Could you check a few things on this drawing? It's one solid part, dimensions in mm from its lowest x, y, z. Give positions to 0.01 mm unless a question says otherwise; leave off trailing zeros. Order: outer loops, then holes, each group sorted by start corner. A loop starts at its lowest first (then second) coordinate and runs counter-clockwise, first axis right, second up. Notation, with made-up numbers: (88, -34.5) -> (101, -34.5) arc R35 cw to (101, 3.5) -> close; hole circle Ø6 at (34.5, 71). An arc over 180 degrees is marked (long way). Answer as CSV lines item,"result".
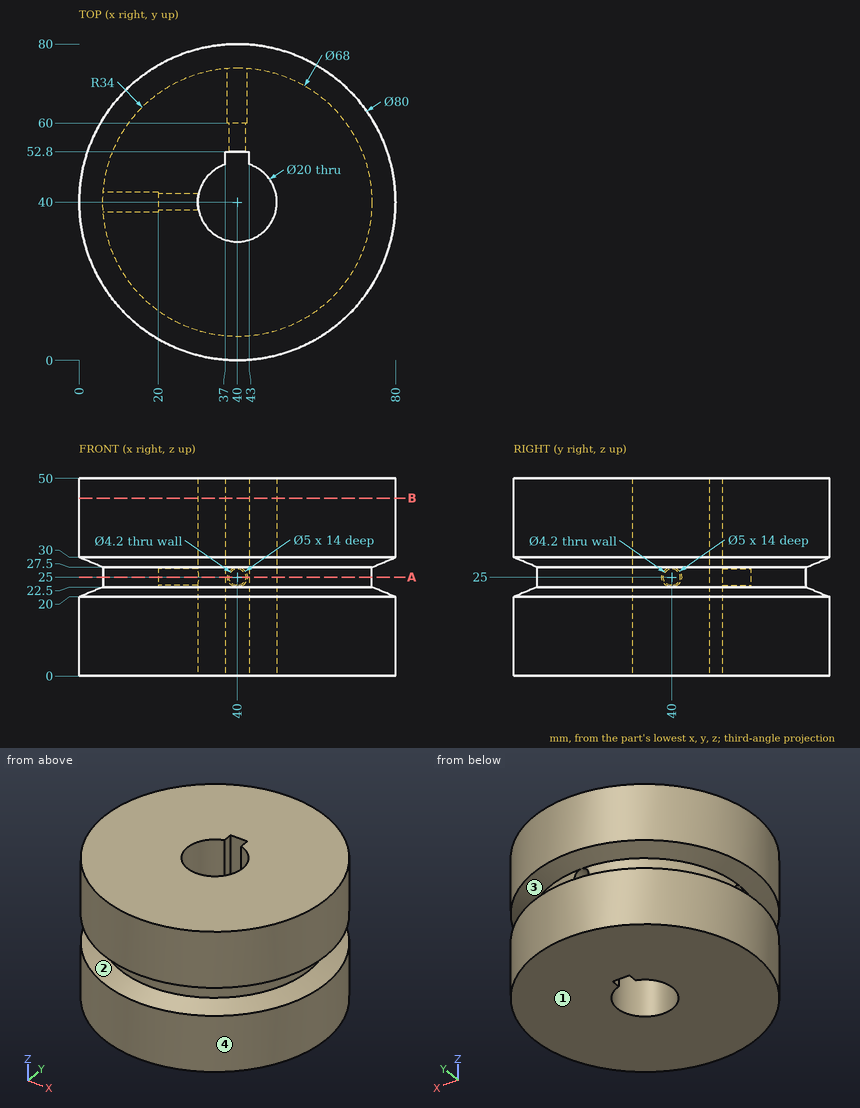
Item 1: Imagine slicing it at A-A, the plane z = 25. Please give me the cut outline in (x, y).
Numbers:
outline,"(6.09, 37.5) arc R34 ccw (long way) to (42.5, 73.91) -> (42.5, 60) -> (42.1, 60) -> (42.1, 52.8) -> (43, 52.8) -> (43, 49.54) arc R10 cw (long way) to (30.22, 37.9) -> (20, 37.9) -> (20, 37.5) -> close; (6.09, 42.5) -> (20, 42.5) -> (20, 42.1) -> (30.22, 42.1) arc R10 cw to (37, 49.54) -> (37, 52.8) -> (37.9, 52.8) -> (37.9, 60) -> (37.5, 60) -> (37.5, 73.91) arc R34 ccw to start"
Item 2: Imagine slicing it at B-B, the plane z = 45. Please give me the cut outline in (x, y).
Numbers:
outline,"circle Ø80 at (40, 40); hole (37, 49.54) arc R10 ccw (long way) to (43, 49.54) -> (43, 52.8) -> (37, 52.8) -> close"
Item 3: We'd pull the mould along Z, two halves only. Please class the marked faces 1, 2, 3 and 4: released by +Z, released by -Z, zero draft, split by the parting line, or undercut.
Numbers:
face 1,"released by -Z"
face 2,"undercut"
face 3,"undercut"
face 4,"zero draft"
Item 4: Please list where these lines run through material, in increasing order: line 1 along X through (y, z) = (40, 38.5); line 2 along Z through (x, y) = (40, 58); line 3 along Z through (x, y) = (40, 63).
Numbers:
line 1,"x = 0 to 30, 50 to 80"
line 2,"z = 0 to 22.9, 27.1 to 50"
line 3,"z = 0 to 22.5, 27.5 to 50"
Item 5: For pin 1 (4 mm diameter, centred on x = 40.5, z = 26, fed in from +Y); pin 2 (1.5 mm diameter, centred on x = 23.5, z = 18.5, fed in from -Y); pin 3 (5 mm diameter, centred on y = 61, z = 9.5, fed in from +X), each with a flat end and sliding along its axis, tell me the tip position at first contact or that it passes through.
Numbers:
pin 1,"stops at y = 75.2"
pin 2,"stops at y = 3.23"
pin 3,"stops at x = 75.46"
